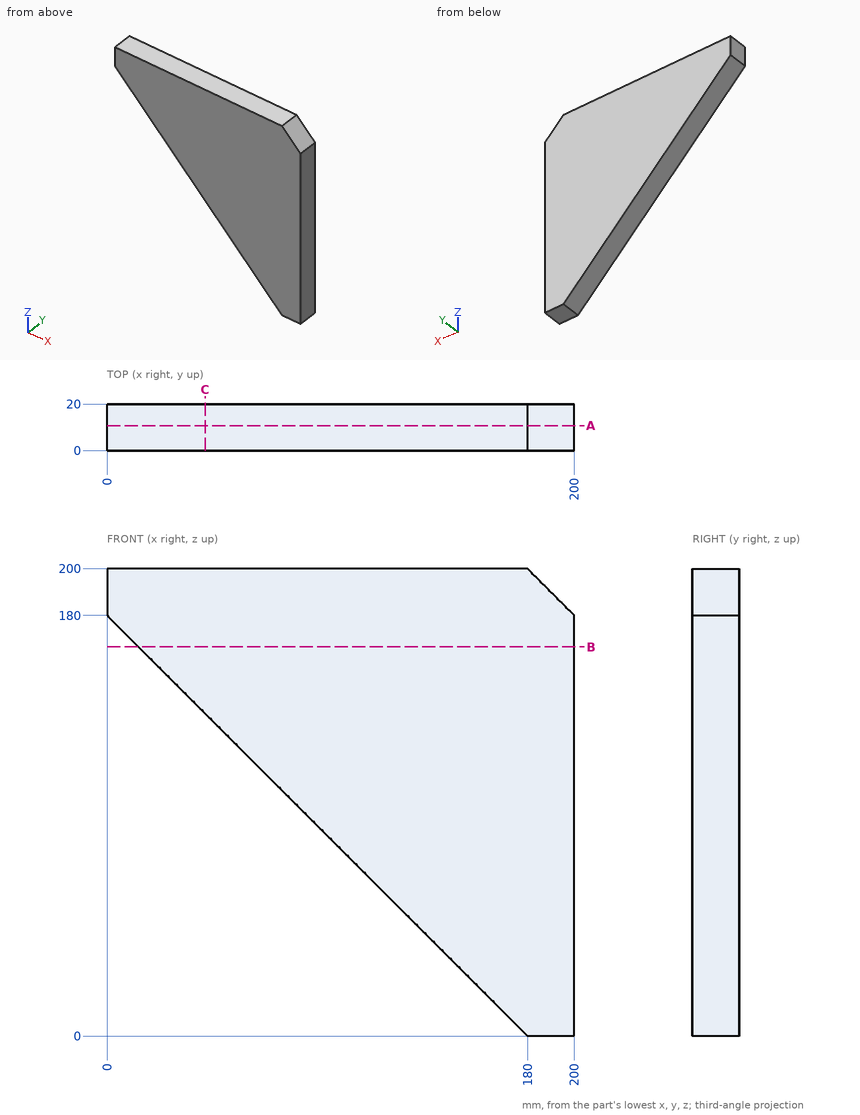
Study the drawing (mm; zero at the part's minimum x, y, z) and answer. Round coordinates to 2 decimals unless told otherwise and drop trailing zeros. Loops run counter-clockwise (first coordinate to the right, second up) from the corner with the lowest first, then second, coordinate; pieces in that order, holes last. Notation, with made-up numbers: (35, 48.5) -> (59, 48.5) arc R26 ccw to (59, 78.5) -> close; hole circle Ø2 at (31.5, 2). An arc over 180 degrees is marked (long way). One line per item, written item: value.
1) Consider L1, parallel to Z at x = 110, y = 4.5; L2, parallel to Z at x = 101, y = 18.5; L3, parallel to X at y = 14.5, z = 88. Determine where each line is inside the solid, lowest interval first. Write a range as [from, to].
Answer list:
L1: z = [70, 200]
L2: z = [79, 200]
L3: x = [92, 200]
2) A cutting plane is placed at A-A (y = 10.75). Determine the outline of the cut face in (x, z).
Answer list:
outline: (0, 180) -> (180, 0) -> (200, 0) -> (200, 180) -> (180, 200) -> (0, 200) -> close
3) A cutting plane is placed at B-B (z = 166.5). Determine the outline of the cut face in (x, y), and give its area (3 significant figures).
Answer list:
outline: (13.5, 0) -> (200, 0) -> (200, 20) -> (13.5, 20) -> close
area: 3,730 mm²
4) A cutting plane is placed at C-C (x = 42). Determine the outline of the cut face in (y, z), and give its area (3 significant figures).
Answer list:
outline: (0, 138) -> (20, 138) -> (20, 200) -> (0, 200) -> close
area: 1,240 mm²
5) Flat-ended cylindrical pins translate along their axes: P1, Ø3, axis at y = 6, z = 173, coming from the -X side; P2, Ø6, axis at x = 168.5, y = 14.5, coming from the -Z side. Find the tip coordinate at first contact, or state that the pin passes through.
Answer list:
P1: stops at x = 5.5
P2: stops at z = 8.5
